```python
from build123d import *

# Parameters (mm, degrees)
MEMBER_4X4_1_DEPTH = 299


with BuildPart() as part:
    # Sketch13 → Member 4X4_1 (new body)
    with BuildSketch(Plane(origin=(0, 0, 0), x_dir=(0, 0, -1), z_dir=(1, 0, 0))):
        with BuildLine():
            Line((40, 0), (0, 0))
            Line((0, 0), (0, -40))
            Line((0, -40), (2.666666667, -40))
            ThreePointArc((2.666666667, -40), (3.609475708, -39.609475708), (4, -38.666666667))
            Line((4, -38.666666667), (4, -9))
            ThreePointArc((4, -9), (5.464466094, -5.464466094), (9, -4))
            Line((9, -4), (38.666666667, -4))
            ThreePointArc((38.666666667, -4), (39.609475708, -3.609475708), (40, -2.666666667))
            Line((40, -2.666666667), (40, 0))
        make_face()
    extrude(amount=MEMBER_4X4_1_DEPTH)


solid = part.part
```
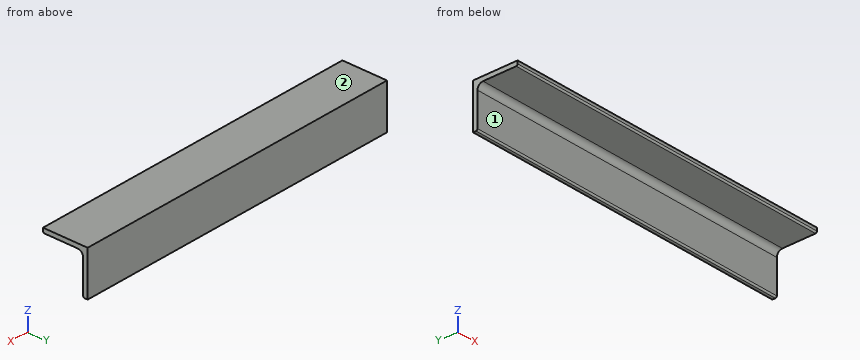
CAD build for the part. Positions are in the model's coordinates, mm. Face numbers are marked on the shaded views. A direction names the side the tool comes from. Give positions to 0.01 mm unless a question says otherwise; leave off trailing zeros. Loops run counter-clockwise (first coordinate to the right, second up) from the corner with the lowest first, then second, coordinate; pieces in that order, holes last. Notation, with made-up numbers: M 82.25,86.5 L 88.25,86.5 A24 ccw 88.25,118.5 Z; hole C -14.5,84 d7. An arc over 180 degrees is marked long. Use one line per item in the form item = value.
Item 1: Drill centre lines: probe 1 along Y at (x, z) = (103, -22.5); probe 2 along Z at (x, y) = (253, -4.5). Where is each one in solid material? Low to high. Write a range as from..to.
Determined:
probe_1 = -4..0
probe_2 = -6.82..0
Item 2: Slice it at A-A (x = 41). List the corners of the cut face in (y, z).
Determined:
outline = M -40,-2.67 A1.33 ccw -38.67,-4 L -9,-4 A5 cw -4,-9 L -4,-38.67 A1.33 ccw -2.67,-40 L 0,-40 L 0,0 L -40,0 Z
Item 3: Slice it at B-B (z = -26). List the corners of the cut face in (x, y).
Determined:
outline = M 0,-4 L 299,-4 L 299,0 L 0,0 Z
Item 4: Flat gauge pins, fed straight in: pin 1 (10 mm diameter, centred on y = -13.5, z = -34.5, fed in from -X); pin 2 (8 mm diameter, centred on x = 223, y = -34.5, fed in from +Z); pin 3 (9 mm diameter, centred on x = 128, y = -31, fed in from -Z); pin 4 (23.5 mm diameter, centred on x = 136, z = -22.5, fed in from -Y). Where does each tip first touch, or does it go through?
Determined:
pin_1 = through
pin_2 = 0
pin_3 = -4
pin_4 = -4
Item 5: Which spindle directions (+Z, -Z, +X, -X, +Y, -Y) get a long thin tool onto all of the face, cutting with end or side? Do the marked faces 1 and 2. Say none if no direction does.
Determined:
face_1 = -Z, +X, -X, -Y
face_2 = +Z, +X, -X, +Y, -Y
